```python
from build123d import *

# Parameters (mm, degrees)
EXTRUDE_1_DEPTH     = 571
SHELL_1_T           = -2
SKETCH_2_W          = 30
SKETCH_2_H          = 1142
EXTRUDE_2_DEPTH     = 2
SKETCH_3_R          = 4.5
CUT_EXTRUDE_1_DEPTH = 1175
EXTRUDE_3_DEPTH     = 2
SKETCH_6_R          = 4.5
CUT_EXTRUDE_2_DEPTH = 2
SKETCH_7_R          = 4.5
CUT_EXTRUDE_3_DEPTH = 10


with BuildPart() as part:
    # 草图1 → 凸台-拉伸1 (new, symmetric)
    with BuildSketch(Plane.XY):
        Polygon((0, 0), (-813, 0), (-813, 30), (-713.029639528, 100), (0, 100), align=None)
    extrude(amount=EXTRUDE_1_DEPTH, both=True)

    # 抽壳1
    shell_1_openings = [part.faces().sort_by_distance(p)[0] for p in [
        (-406.5, 0, 0),
    ]]
    offset(amount=SHELL_1_T, openings=shell_1_openings, kind=Kind.INTERSECTION)

    # 草图2 → 凸台-拉伸2 (add)
    with BuildSketch(Plane.XZ):
        with Locations((13, 0)):
            Rectangle(SKETCH_2_W, SKETCH_2_H)
    extrude(amount=-EXTRUDE_2_DEPTH)

    # 草图3 → 切除-拉伸1 (cut)
    with BuildSketch(Plane.XY.offset(571)):
        with Locations((-683.029639528, 84)):
            Circle(SKETCH_3_R)
        with Locations((-30, 84)):
            Circle(SKETCH_3_R)
    extrude(amount=-CUT_EXTRUDE_1_DEPTH, mode=Mode.SUBTRACT)

    # 草图5 → 凸台-拉伸3 (add)
    with BuildSketch(Plane.XZ):
        Polygon((-783, 541), (0, 541), (0, 571), (-813, 571), (-813, -571), (0, -571), (0, -541), (-783, -541), align=None)
    extrude(amount=-EXTRUDE_3_DEPTH)

    # 草图6 → 切除-拉伸2 (cut)
    with BuildSketch(Plane.XZ):
        with Locations((-797, 541)):
            Circle(SKETCH_6_R)
        with Locations((-797, -541)):
            Circle(SKETCH_6_R)
        with Locations((-797, 0)):
            Circle(SKETCH_6_R)
    extrude(amount=-CUT_EXTRUDE_2_DEPTH, mode=Mode.SUBTRACT)

    # 草图7 → 切除-拉伸3 (cut)
    with BuildSketch(Plane(origin=(0, 0, 0), x_dir=(0, 0, -1), z_dir=(1, 0, 0))):
        with Locations((-555, 84)):
            Circle(SKETCH_7_R)
        with Locations((-487, 84)):
            Circle(SKETCH_7_R)
    extrude(amount=-CUT_EXTRUDE_3_DEPTH, mode=Mode.SUBTRACT)


solid = part.part
```
Work out the finished part from the listing and answer in its coordinate system (mm). A direction names the side the tool comes from. Round coordinates to 2 decimals unless told otherwise and drop trailing zeros. Loops run counter-clockwise (first coordinate to the right, second up) from the corner with the lowest first, then second, coordinate; pieces in that order, holes last.
(1) For faces 4 (the flat face through (-401, 51, -569)), 5 (the flat face through (-813, 15, 8)), 6 (the flat face through (14, 2, 8)), determine the directions among +Z, -Z, +X, -X, +Y, -Y from which every point of the face is accessible in a straight line to the end or side of a thin tool.
Computed values:
face 4: none
face 5: +Z, -Z, -X, +Y, -Y
face 6: +Z, -Z, +X, +Y
(2) The mould has two halves that part along X. Classify faces 1 (the flat face through (-387, 51, -571)), 2 (the flat face through (-811, 15, 8)), 3 (the flat face through (0, 52, 8)): pulls with the +X half, pulls with the -X half, needs draft (parallel to the pull), parting line crosses it, or undercut.
Computed values:
face 1: needs draft
face 2: undercut
face 3: pulls with the +X half
(3) The part is cut by section C-C, the plane y = 63. Give the vertices of the cut face in (x, z), and give its area (3 significant figures).
Computed values:
outline: (-765.87, -571) - (0, -571) - (0, 571) - (-765.87, 571) - close; hole (-762.38, -569) - (-2, -569) - (-2, 569) - (-762.38, 569) - close
area: 9,310 mm2
(4) The part is cut by section A-A, the plane z = 370.5. Give the vertices of the cut face in (x, y).
Computed values:
outline: (-813, 0) - (-783, 0) - (-783, 2) - (-811, 2) - (-811, 28.96) - (-712.4, 98) - (-2, 98) - (-2, 0) - (28, 0) - (28, 2) - (0, 2) - (0, 100) - (-713.03, 100) - (-813, 30) - close
(5) Each of these flat-tipped pins is pushed along its axis until it touches: P1, Ø7, axis at y = 84, z = 487, coming from the +X side; P2, Ø1, axis at x = -418, z = -31, coming from the -Y side; P3, Ø5.5, axis at x = -797, z = -541, coming from the -Y side. Where does it stop, or does it pass through?
Computed values:
P1: stops at x = -727.39
P2: stops at y = 98
P3: stops at y = 36.84
(6) The part is cut by section B-B, the plane x = -544.5. Give the vertices of the cut face in (y, z).
Computed values:
outline: (0, -571) - (100, -571) - (100, 571) - (0, 571) - (0, 541) - (2, 541) - (2, 569) - (98, 569) - (98, -569) - (2, -569) - (2, -541) - (0, -541) - close
(7) Find the intervals of material crossed by L1, parallel to Z at x = -797, y = 1; L2, parallel to Z at x = -522.5, y = 88; L3, parallel to X at y = 23, z = 454.5, in increasing order.
Computed values:
L1: z = -571 to -545.5, -536.5 to -4.5, 4.5 to 536.5, 545.5 to 571
L2: z = -571 to -569, 569 to 571
L3: x = -813 to -811, -2 to 0
(8) The part is cut by section D-D, the plane x = -746.5. Give the vertices of the cut face in (y, z), and give its area (3 significant figures).
Computed values:
outline: (0, -571) - (76.56, -571) - (76.56, 571) - (0, 571) - (0, 541) - (2, 541) - (2, 569) - (74.12, 569) - (74.12, -569) - (2, -569) - (2, -541) - (0, -541) - close
area: 3,200 mm2
